```python
from build123d import *

# Parameters (mm, degrees)
BASE_PLATE_DEPTH           = 12
BASE_PROFILE_CUT_SKETCH_W  = 10
BASE_PROFILE_CUT_SKETCH_H  = 6
BASE_PROFILE_CUT_DEPTH     = 60
SIDE_NOTCH_SKETCH_W        = 13
SIDE_NOTCH_SKETCH_H        = 12
SIDE_NOTCH_CUT_DEPTH       = 60
UPRIGHT_WEB_SKETCH_W       = 12
UPRIGHT_WEB_SKETCH_H       = 60
UPRIGHT_WEB_DEPTH          = 12
LUG_BLOCK_SKETCH_W         = 12
LUG_BLOCK_SKETCH_H         = 13
LUG_BLOCK_DEPTH            = 60
WEB_PAD_SKETCH_W           = 12
WEB_PAD_SKETCH_H           = 60
WEB_PAD_1MM_DEPTH          = 1
EAR_BASE_DEPTH             = 12
UPPER_CLEVIS_LUG_DEPTH     = 7.5
LOWER_START                = -7.5
LOWER_CLEVIS_LUG_DEPTH     = 7.5
CLEVIS_SPACER_SKETCH_W     = 13
CLEVIS_SPACER_SKETCH_H     = 45
CLEVIS_SPACER_BLOCK_DEPTH  = 28
LUG_PAD_SKETCH_W           = 28
LUG_PAD_SKETCH_H           = 45
LUG_PAD_5MM_DEPTH          = 5
CLEVIS_SLOT_CUT_DEPTH      = 12
HOLE_10_SKETCH_R           = 5
HOLE_10_DEPTH              = 60
UPPER_PIN_HOLE_18_SKETCH_R = 9
UPPER_PIN_HOLE_18_DEPTH    = 60
LOWER_PIN_HOLE_18_SKETCH_R = 9
LOWER_PIN_HOLE_18_DEPTH    = 60
EAR_ROUND_CUT_DEPTH        = 60
EAR_BOSS_SKETCH_W          = 12
EAR_BOSS_SKETCH_H          = 60
EAR_BOSS_7MM_DEPTH         = 7
EAR_PLATE_DEPTH            = 12
EAR_BORE_16_SKETCH_R       = 8
EAR_BORE_16_DEPTH          = 12
EAR_START                  = -4
EAR_RELIEF_CUT_A_DEPTH     = 4
EAR_RELIEF_CUT_B_DEPTH     = 4


with BuildPart() as part:
    # Base Plate Sketch → Base Plate (new body)
    with BuildSketch(Plane.XY):
        Polygon((0, 0), (50, 0), (63, 0), (63, 60), (50, 60), (0, 60), align=None)
    extrude(amount=BASE_PLATE_DEPTH)

    # Base Profile Cut Sketch → Base Profile Cut (cut)
    with BuildSketch(Plane.XZ):
        with Locations((5, 9)):
            Rectangle(BASE_PROFILE_CUT_SKETCH_W, BASE_PROFILE_CUT_SKETCH_H)
    extrude(amount=-BASE_PROFILE_CUT_DEPTH, mode=Mode.SUBTRACT)

    # Side Notch Sketch → Side Notch Cut (cut)
    with BuildSketch(Plane.XZ):
        with Locations((56.5, 6)):
            Rectangle(SIDE_NOTCH_SKETCH_W, SIDE_NOTCH_SKETCH_H)
    extrude(amount=-SIDE_NOTCH_CUT_DEPTH, mode=Mode.SUBTRACT)

    # Upright Web Sketch → Upright Web (add)
    with BuildSketch(Plane.XY.offset(12)):
        with Locations((56, 30)):
            Rectangle(UPRIGHT_WEB_SKETCH_W, UPRIGHT_WEB_SKETCH_H)
    extrude(amount=-UPRIGHT_WEB_DEPTH)

    # Lug Block Sketch → Lug Block (add)
    with BuildSketch(Plane.XZ):
        with Locations((44, 18.5)):
            Rectangle(LUG_BLOCK_SKETCH_W, LUG_BLOCK_SKETCH_H)
    extrude(amount=-LUG_BLOCK_DEPTH)

    # Web Pad Sketch → Web Pad 1mm (add)
    with BuildSketch(Plane(origin=(62, 0, 0), x_dir=(0, 0, -1), z_dir=(1, 0, 0))):
        with Locations((-6, 30)):
            Rectangle(WEB_PAD_SKETCH_W, WEB_PAD_SKETCH_H)
    extrude(amount=WEB_PAD_1MM_DEPTH)

    # Ear Base Sketch → Ear Base (add)
    with BuildSketch(Plane.XY.offset(12)):
        with BuildLine():
            Line((63, 60), (63, 0))
            ThreePointArc((63, 0), (93, 30), (63, 60))
        make_face()
    extrude(amount=-EAR_BASE_DEPTH)

    # Upper Clevis Lug Sketch → Upper Clevis Lug (add)
    with BuildSketch(Plane.XZ):
        with BuildLine():
            Line((38, 59.358797437), (38, 25))
            Line((38, 25), (38, 12))
            Line((38, 12), (10, 12))
            Line((10, 12), (10, 35.694478304))
            ThreePointArc((10, 35.694478304), (-1.491933385, 77.689100216), (38, 59.358797437))
        make_face()
    extrude(amount=-UPPER_CLEVIS_LUG_DEPTH)

    # Lower Clevis Lug Sketch → Lower Clevis Lug (add)
    with BuildSketch(Plane(origin=(0, 60, 0), x_dir=(1, 0, 0), z_dir=(0, 1, 0)).offset(LOWER_START)):
        with BuildLine():
            Line((38, -12), (38, -59.358797437))
            ThreePointArc((38, -59.358797437), (-1.491933385, -77.689100216), (10, -35.694478304))
            Line((10, -35.694478304), (10, -12))
            Line((10, -12), (38, -12))
        make_face()
    extrude(amount=LOWER_CLEVIS_LUG_DEPTH)

    # Clevis Spacer Sketch → Clevis Spacer Block (add)
    with BuildSketch(Plane.ZY.offset(-38)):
        with Locations((18.5, 30)):
            Rectangle(CLEVIS_SPACER_SKETCH_W, CLEVIS_SPACER_SKETCH_H)
    extrude(amount=CLEVIS_SPACER_BLOCK_DEPTH)

    # Lug Pad Sketch → Lug Pad 5mm (add)
    with BuildSketch(Plane.XY.offset(25)):
        with Locations((24, 30)):
            Rectangle(LUG_PAD_SKETCH_W, LUG_PAD_SKETCH_H)
    extrude(amount=LUG_PAD_5MM_DEPTH)

    # Clevis Slot Sketch → Clevis Slot Cut (cut)
    with BuildSketch(Plane(origin=(50, 0, 0), x_dir=(0, 0, -1), z_dir=(1, 0, 0))):
        with BuildLine():
            Line((-25, 42.5), (-25, 17.5))
            ThreePointArc((-25, 17.5), (-12.5, 30), (-25, 42.5))
        make_face()
    extrude(amount=-CLEVIS_SLOT_CUT_DEPTH, mode=Mode.SUBTRACT)

    # Hole Ø10 Sketch → Hole Ø10 (cut)
    with BuildSketch(Plane.XZ):
        with Locations(Location((23, 12, 0), (0, 0, 270))):
            Circle(HOLE_10_SKETCH_R)
    extrude(amount=-HOLE_10_DEPTH, mode=Mode.SUBTRACT)

    # Upper Pin Hole Ø18 Sketch → Upper Pin Hole Ø18 (cut)
    with BuildSketch(Plane.XZ):
        with Locations(Location((14, 59.358797437, 0), (0, 0, 270))):
            Circle(UPPER_PIN_HOLE_18_SKETCH_R)
    extrude(amount=-UPPER_PIN_HOLE_18_DEPTH, mode=Mode.SUBTRACT)

    # Lower Pin Hole Ø18 Sketch → Lower Pin Hole Ø18 (cut)
    with BuildSketch(Plane.XY.offset(30)):
        with Locations((24, 30)):
            Circle(LOWER_PIN_HOLE_18_SKETCH_R)
    extrude(amount=-LOWER_PIN_HOLE_18_DEPTH, mode=Mode.SUBTRACT)

    # Ear Round Cut Sketch → Ear Round Cut (cut)
    with BuildSketch(Plane.XY.offset(12)):
        with BuildLine():
            Line((63, 60), (63, 0))
            ThreePointArc((63, 0), (93, 30), (63, 60))
        make_face()
    extrude(amount=-EAR_ROUND_CUT_DEPTH, mode=Mode.SUBTRACT)

    # Ear Boss Sketch → Ear Boss 7mm (add)
    with BuildSketch(Plane(origin=(63, 0, 0), x_dir=(0, 0, -1), z_dir=(1, 0, 0))):
        with Locations((-6, 30)):
            Rectangle(EAR_BOSS_SKETCH_W, EAR_BOSS_SKETCH_H)
    extrude(amount=EAR_BOSS_7MM_DEPTH)

    # Ear Plate Sketch → Ear Plate (add)
    with BuildSketch(Plane.XY.offset(12)):
        with BuildLine():
            Line((70, 60), (70, 0))
            ThreePointArc((70, 0), (100, 30), (70, 60))
        make_face()
    extrude(amount=-EAR_PLATE_DEPTH)

    # Ear Bore Ø16 Sketch → Ear Bore Ø16 (cut)
    with BuildSketch(Plane.XY.offset(12)):
        with Locations((70, 30)):
            Circle(EAR_BORE_16_SKETCH_R)
    extrude(amount=-EAR_BORE_16_DEPTH, mode=Mode.SUBTRACT)

    # Ear Relief A Sketch → Ear Relief Cut A (cut)
    with BuildSketch(Plane(origin=(0, 0, 0), x_dir=(-1, 0, 0), z_dir=(0, 0, -1)).offset(EAR_START)):
        with BuildLine():
            Line((-93.315470525, 48.878263537), (-93.315470525, 11.121736463))
            ThreePointArc((-93.315470525, 11.121736463), (-100, 30), (-93.315470525, 48.878263537))
        make_face()
    extrude(amount=EAR_RELIEF_CUT_A_DEPTH, mode=Mode.SUBTRACT)

    # Ear Relief B Sketch → Ear Relief Cut B (cut)
    with BuildSketch(Plane(origin=(0, 0, 0), x_dir=(-1, 0, 0), z_dir=(0, 0, -1)).offset(EAR_START)):
        with BuildLine():
            Line((-89.315470525, 7.045423149), (-89.315470525, 30))
            Line((-89.315470525, 30), (-89.315470525, 52.954576851))
            ThreePointArc((-89.315470525, 52.954576851), (-91.41269171, 51.011821285), (-93.315470525, 48.878263537))
            Line((-93.315470525, 48.878263537), (-93.315470525, 11.121736463))
            ThreePointArc((-93.315470525, 11.121736463), (-91.41269171, 8.988178715), (-89.315470525, 7.045423149))
        make_face()
    extrude(amount=EAR_RELIEF_CUT_B_DEPTH, mode=Mode.SUBTRACT)


solid = part.part
```
The model under review builds one solid part; all positions refer to its coordinate system, in mm. A direction names the side the tool comes from. Round coordinates to 2 decimals unless told otherwise and drop trailing zeros. Write each loop counter-clockwise with the first axis right and the second up, starting at its lowest first coordinate (ties: lowest second). Pieces come first, ordered by that corner, then holes.
(1) We need section B-B on y = 30. Give the boundary of the cut face in (x, z), and give its area (3 significant figures).
(2) Insertion check: pin 1 (8 mm diameter, centred on x = 4, y = 33.5, fed in from +Z); pin 2 (2 mm diameter, centred on y = 21.5, z = 1.5, fed in from +X); pin 3 (10 mm diameter, centred on x = 44, y = 35.5, fed in from +Z). Each pin has a flat end and moves straight along its axis. Give the tip position at first contact, or say it passes through.
(3) Wall thickness on L1, parallel to Z at x = 23.5, y = 13; L2, parallel to Y at x = -3, z = 54; L3, parallel to X at y = 42.5, z = 12.5: over which ranges is each line inside the solid? List them lowest first.
(4) Mouldability with a two-part tool opening along Y and no side actions: class faces 5 (the cylindrical face through (-0.901, 56.198, 78.173)), 6 (the cylindrical face through (64.1, 35.4, 6.1)), 7 (the cylindrical face through (99.993, 29.34, 7.417)) as +Y half, -Y half, draft (parallel to the pull), parting line (faces both ways), or undercut.
(5) We need section A-A on z = 33.5. Give the boundary of the cut face in (x, y).
(6) We need section C-C on x = 68.5. Give the boundary of the cut face in (y, z).
(7) We need section D-D on z = 20. Give the boundary of the cut face in (x, y).
(8) Machinability: for faces 1 (the flat face through (44, 9, 25)), 2 (the flat face through (94, 30, 4)), 3 (the flat face through (5, 30, 6)), 4 (the flat face through (20, 7.5, 51)), which of the approach directions +Z, -Z, +X, -X, +Y, -Y give a long, thin tool a straight path to every point of the face, cutting with its end or side? Answer none if there is none.
Findings below:
1. outline: (0, 0) - (15, 0) - (15, 30) - (10, 30) - (10, 6) - (0, 6) - close; (33, 0) - (62, 0) - (62, 12) - (50, 12) - (50, 12.5) - (38, 12.5) - (38, 30) - (33, 30) - close; (78, 0) - (89.32, 0) - (89.32, 4) - (100, 4) - (100, 12) - (78, 12) - close
1. area: 875 mm2
2. pin 1: stops at z = 6
2. pin 2: stops at x = 89.32
2. pin 3: stops at z = 18.22
3. L1: z = 0 to 7.03, 16.97 to 30
3. L2: y = 0 to 7.5, 52.5 to 60
3. L3: x = 10 to 18.03, 27.97 to 50
4. face 5: draft
4. face 6: undercut
4. face 7: parting line
5. outline: (10, 0) - (38, 0) - (38, 7.5) - (10, 7.5) - close; (10, 52.5) - (38, 52.5) - (38, 60) - (10, 60) - close
6. outline: (0, 0) - (22.14, 0) - (22.14, 12) - (0, 12) - close; (37.86, 0) - (60, 0) - (60, 12) - (37.86, 12) - close
7. outline: (10, 0) - (50, 0) - (50, 18.54) - (38, 18.54) - (38, 41.46) - (50, 41.46) - (50, 60) - (10, 60) - close; hole circle Ø18 at (24, 30)
8. face 1: +Z, +X, +Y, -Y
8. face 2: -Z, +X, +Y, -Y
8. face 3: -X, +Y, -Y
8. face 4: +Z, +X, -X
